Design review of the part built by this model. Coordinates are the model's own, in mm. Face numbers are marked on the shaded views. A direction names the side the tool comes from. Round coordinates to 2 decimals unless told otherwise and drop trailing zeros. Loops run counter-clockwise (first coordinate to the right, second up) from the corner with the lowest first, then second, coordinate; pieces in that order, holes last. Notation, with made-up numbers: (-14.5, 79.5) - (34.5, 79.5) arc R31 cw to (34.5, 115.5) - close; hole circle Ø1 at (5.5, -30.75). An arc over 180 degrees is marked (long way). Use one line per item in the form item = value. Start each with the question number.
(1) For pin 1 (12 mm diameter, centred on y = 0, z = 0, fed in from +X); pin 2 (1.5 mm diameter, centred on y = -11, z = -12, fed in from -X); pin 3 (5 mm diameter, centred on x = 8, y = 11, fed in from +Z); pin 4 (1.5 mm diameter, centred on x = 7, y = 6, fed in from +Z), all flat-tipped, find the tip position at first contact; note any pin that passes through.
(2) We need section C-C, the plane x = 5. Write out the cut boundary in (y, z).
(3) Machinability: for the marked faces 1 and 2, which of the approach directions +Z, -Z, +X, -X, +Y, -Y give a long, thin tool a straight path to every point of the face, cutting with its end or side? Answer none if there is none.
(4) We need section A-A, the plane y = 0. Write out the cut boundary in (x, z).
(5) The part is to be moulded in two halves that separate along Z. For the marked faces 3, 4 and 5, say which applies: released by +Z, released by -Z, zero draft, split by the parting line, or undercut.
(6) We need section B-B, the plane z = 0. Write out the cut boundary in (x, y), then the cut area to 3 significant figures.
(7) Wall thickness on probe 1 along Y at (x, z) = (2.25, 0); probe 2 along X at (y, z) = (13.5, -4); probe 3 along Z at (x, y) = (5, 11.5): over which ranges is each line inside the solid? List them lowest first. Write a range as [from, to].
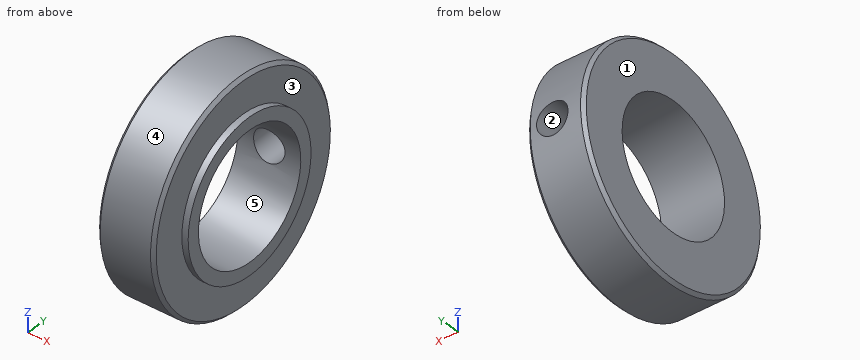
from build123d import *

# Parameters (mm, degrees)
M6_TAPPED_HOLE1_D               = 5
M6_TAPPED_HOLE1_DEPTH           = 15
M6_TAPPED_HOLE1_TIP             = 1.502151548
M6_TAPPED_HOLE1_ON_FACE_2_D     = 5
M6_TAPPED_HOLE1_ON_FACE_2_DEPTH = 15
M6_TAPPED_HOLE1_ON_FACE_2_TIP   = 1.502151548
CHAMFER1_SIZE                   = 0.5


with BuildPart() as part:
    # Sketch1 → Revolve1 (revolve)
    with BuildSketch(Plane.XY, mode=Mode.PRIVATE) as revolve1_sk:
        Polygon((0, 10), (10, 10), (10, 12), (9, 12), (9, 17.5), (0, 17.5), align=None)
    revolve(revolve1_sk.sketch.rotate(Axis((0, 0, 0), (1, 0, 0)), 90), axis=Axis((0, 0, 0), (1, 0, 0)))

    # M6 Tapped Hole1
    with Locations(Plane(origin=(5, 17.5, 0), x_dir=(0, 0, 1), z_dir=(0, 1, 0))):
        with Locations((0, 0)):
            Hole(M6_TAPPED_HOLE1_D / 2, depth=M6_TAPPED_HOLE1_DEPTH)
            with Locations((0, 0, -(M6_TAPPED_HOLE1_DEPTH + M6_TAPPED_HOLE1_TIP / 2))):  # 118° drill point
                Cone(0, M6_TAPPED_HOLE1_D / 2, M6_TAPPED_HOLE1_TIP, mode=Mode.SUBTRACT)

    # M6 Tapped Hole1 on face 2
    with Locations(Plane(origin=(-19.39268328, -13.895465991, 0), x_dir=(0, 0, 1), z_dir=(0, 1, 0))):
        with Locations((0, 0)):
            Hole(M6_TAPPED_HOLE1_ON_FACE_2_D / 2, depth=M6_TAPPED_HOLE1_ON_FACE_2_DEPTH)
            with Locations((0, 0, -(M6_TAPPED_HOLE1_ON_FACE_2_DEPTH + M6_TAPPED_HOLE1_ON_FACE_2_TIP / 2))):  # 118° drill point
                Cone(0, M6_TAPPED_HOLE1_ON_FACE_2_D / 2, M6_TAPPED_HOLE1_ON_FACE_2_TIP, mode=Mode.SUBTRACT)

    # Chamfer1
    chamfer1_edges = [part.edges().sort_by_distance(p)[0] for p in [
        (9, 0, -17.5),
        (0, 0, -17.5),
    ]]
    chamfer(chamfer1_edges, length=CHAMFER1_SIZE)


solid = part.part
Data:
q1.pin_1 = through
q1.pin_2 = 0
q1.pin_3 = 15.3
q1.pin_4 = 16.69
q2.outline = (9.68, -2.5) arc R10 cw (long way) to (9.68, 2.5) - (17.32, 2.5) arc R17.5 ccw (long way) to (17.32, -2.5) - close
q3.face_1 = +Z, -Z, -X, +Y, -Y
q3.face_2 = +Y
q4.outline = (0, -17) - (0.5, -17.5) - (8.5, -17.5) - (9, -17) - (9, -12) - (10, -12) - (10, -10) - (0, -10) - close; (0, 10) - (10, 10) - (10, 12) - (9, 12) - (9, 17) - (8.5, 17.5) - (0.5, 17.5) - (0, 17) - close
q5.face_3 = zero draft
q5.face_4 = split by the parting line
q5.face_5 = undercut
q6.outline = (0, -17) - (0.5, -17.5) - (8.5, -17.5) - (9, -17) - (9, -12) - (10, -12) - (10, -10) - (0, -10) - close; (0, 10) - (2.5, 10) - (2.5, 17.5) - (0.5, 17.5) - (0, 17) - close; (7.5, 10) - (10, 10) - (10, 12) - (9, 12) - (9, 17) - (8.5, 17.5) - (7.5, 17.5) - close
q6.area = 101 mm^2
q7.probe_1 = [-17.5, -10], [10, 17.5]
q7.probe_2 = [0, 9]
q7.probe_3 = [-13.19, -2.5], [2.5, 13.19]
